Can you work these out from the drawing? Everything is in mm from the part's minimum corner. Coordinates: 2 decimals unless noted, no trailing zeros. Loops run counter-clockwise (first coordinate to the right, second up) from the corner with the lowest first, then second, coordinate; pieces in that order, holes last.
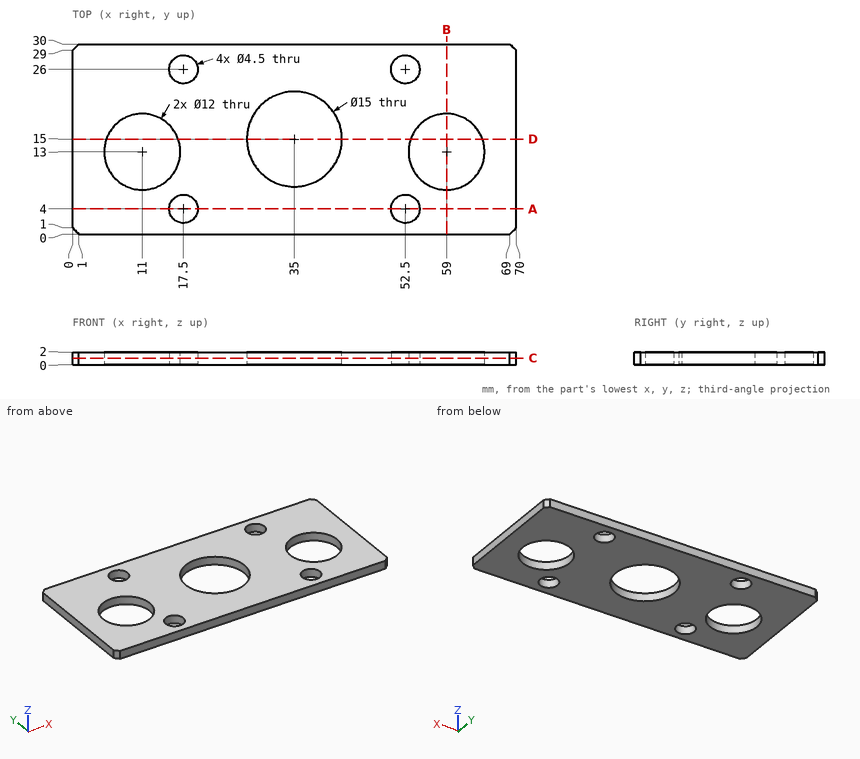
Item 1: Suppose I cut it at D-D, the plane y = 15. Please give me the cut outline in (x, z), plus the area to 3 significant figures.
Results are:
outline: (0, 0) - (5.34, 0) - (5.34, 2) - (0, 2) - close; (16.66, 0) - (27.5, 0) - (27.5, 2) - (16.66, 2) - close; (42.5, 0) - (53.34, 0) - (53.34, 2) - (42.5, 2) - close; (64.66, 0) - (70, 0) - (70, 2) - (64.66, 2) - close
area: 64.7 mm2
Item 2: Suppose I cut it at C-C, the plane z = 1.05. Please give me the cut outline in (x, y).
Results are:
outline: (0, 1) - (1, 0) - (69, 0) - (70, 1) - (70, 29) - (69, 30) - (1, 30) - (0, 29) - close; hole circle Ø12 at (11, 13); hole circle Ø4.5 at (17.5, 4); hole circle Ø4.5 at (17.5, 26); hole circle Ø15 at (35, 15); hole circle Ø4.5 at (52.5, 4); hole circle Ø4.5 at (52.5, 26); hole circle Ø12 at (59, 13)
Item 3: Suppose I cut it at A-A, the plane y = 4. Please give me the cut outline in (x, z), plus the area to 3 significant figures.
Results are:
outline: (0, 0) - (15.25, 0) - (15.25, 2) - (0, 2) - close; (19.75, 0) - (50.25, 0) - (50.25, 2) - (19.75, 2) - close; (54.75, 0) - (70, 0) - (70, 2) - (54.75, 2) - close
area: 122 mm2
Item 4: I need wall thicknesses on line 1 along Y through (x, z) = (17.5, 0.9); line 2 along Y through (x, z) = (35, 0.8); line 3 along Y through (x, z) = (11, 1). Which ranges of each line are inside material? Lowest first, please.
Results are:
line 1: y = 0 to 1.75, 6.25 to 23.75, 28.25 to 30
line 2: y = 0 to 7.5, 22.5 to 30
line 3: y = 0 to 7, 19 to 30
Item 5: Suppose I cut it at B-B, the plane x = 59. Please give me the cut outline in (y, z), plus the area to 3 significant figures.
Results are:
outline: (0, 0) - (7, 0) - (7, 2) - (0, 2) - close; (19, 0) - (30, 0) - (30, 2) - (19, 2) - close
area: 36.0 mm2
Item 6: I'm going to push a flat-ended pin straight in: P1, Ø4, axis at x = 17.5, y = 4, coming from the -Z side. Where does the tip first touch, or does it pass through?
Results are:
P1: passes through
